```python
from build123d import *

# Parameters (mm, degrees)
SKETCH_1_W             = 35
SKETCH_1_H             = 56.7
EXTRUDE_1_DEPTH        = 12
CHAMFER_1_SIZE         = 2
SKETCH_4_W             = 28
SKETCH_4_H             = 12
EXTRUDE_2_DEPTH        = 35
HOLE_WIZARD_M5_1_D     = 4.2
CHAMFER_2_SIZE         = 2
HOLE_WIZARD_M5_2_D     = 4.2
HOLE_WIZARD_M5_2_DEPTH = 12.4
HOLE_WIZARD_M5_2_TIP   = 1.2618073


with BuildPart() as part:
    # 草图1 → 凸台-拉伸1 (new body)
    with BuildSketch(Plane.XY):
        Rectangle(SKETCH_1_W, SKETCH_1_H)
    extrude(amount=EXTRUDE_1_DEPTH)

    # 倒角1
    chamfer_1_edges = [part.edges().sort_by_distance(p)[0] for p in [
        (-17.5, -28.35, 6),
        (17.5, -28.35, 6),
    ]]
    chamfer(chamfer_1_edges, length=CHAMFER_1_SIZE)

    # 草图4 → 凸台-拉伸2 (add)
    with BuildSketch(Plane.ZY.offset(17.5)):
        with Locations((26, 22.35)):
            Rectangle(SKETCH_4_W, SKETCH_4_H)
    extrude(amount=-EXTRUDE_2_DEPTH)

    # M5 螺纹孔1 (through all)
    with Locations(Plane(origin=(0, 0, 0), x_dir=(-1, 0, 0), z_dir=(0, 0, -1))):
        with Locations((-10, -8.35), (10, -8.35)):
            Hole(HOLE_WIZARD_M5_1_D / 2)

    # 倒角2
    chamfer_2_edges = [part.edges().sort_by_distance(p)[0] for p in [
        (-17.5, 22.35, 40),
        (17.5, 22.35, 40),
    ]]
    chamfer(chamfer_2_edges, length=CHAMFER_2_SIZE)

    # M5 螺纹孔2
    with Locations(Plane(origin=(0, 28.35, 0), x_dir=(1, 0, 0), z_dir=(0, 1, 0))):
        with Locations((-10, -6.5), (10, -6.5), (-10, -31.5), (10, -31.5)):
            Hole(HOLE_WIZARD_M5_2_D / 2, depth=HOLE_WIZARD_M5_2_DEPTH)
            with Locations((0, 0, -(HOLE_WIZARD_M5_2_DEPTH + HOLE_WIZARD_M5_2_TIP / 2))):  # 118° drill point
                Cone(0, HOLE_WIZARD_M5_2_D / 2, HOLE_WIZARD_M5_2_TIP, mode=Mode.SUBTRACT)


solid = part.part
```
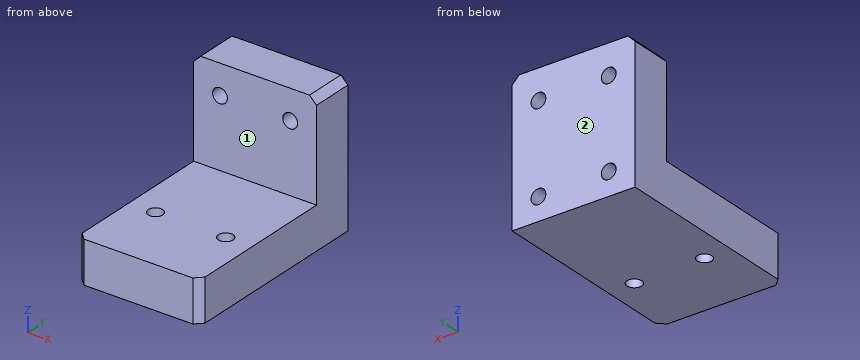
Model file for the job. Use its own axes, mm. Face numbers are marked on the shaded views. A direction names the side the tool comes from. Coordinates: 2 decimals unless noted, no trailing zeros. Loops run counter-clockwise (first coordinate to the right, second up) from the corner with the lowest first, then second, coordinate; pieces in that order, holes last. Notation, with made-up numbers: (67, -10.75) - (100, -10.75) arc R26 ccw to (100, 9.25) - close; hole circle Ø5 at (83.25, -30.5). An arc over 180 degrees is marked (long way). Answer as a JSON object with one key per item and string values. Group by question number.
(1) Cut at A-A (z = 31.5). Give the cut face in (x, y), then the cut area to 3 significant figures.
(2) Cut at B-B (y = -8.35). Give the cut face in (x, z), then the cut area to 3 significant figures.
(3) Cut at D-D (x = -2). Give the cut face in (y, z).
(4) Probe line 1 along Z through (x, y) = (-10, 23); line 2 along Y through (x, z) = (-10, 11.5); line 3 along X through (y, z) = (-8, 8). List the from-to ranges inside material, lowest first.
(5) Flat gauge pins, fed straight in: pin 1 (3.5 mm diameter, centred on x = -10, z = 31.5, fed in from -Y); pin 2 (10 mm diameter, centred on x = -8, z = 35.5, fed in from -Y); pin 3 (4 mm diameter, centred on x = 10, z = 6.5, fed in from +Y); pin 4 (6 mm diameter, centred on x = 14, y = 2.5, fed in from +Z). Where does each tip first touch, or does it go through?
(6) Tool access for the marked faces 1 and 2: list every direction of +Z, -Z, +X, -X, +Y, -Y with a clear straight run to the whole face (end or side of a thin tool).
(7) Cut at C-C (y = 22). Give the cut face in (x, z).
Geometry says:
{
 "1": {"outline": "(-17.5, 16.35) - (-12.1, 16.35) - (-12.1, 28.35) - (-17.5, 28.35) - close; (-7.9, 16.35) - (7.9, 16.35) - (7.9, 28.35) - (-7.9, 28.35) - close; (12.1, 16.35) - (17.5, 16.35) - (17.5, 28.35) - (12.1, 28.35) - close", "area": "319 mm^2"},
 "2": {"outline": "(-17.5, 0) - (-12.1, 0) - (-12.1, 12) - (-17.5, 12) - close; (-7.9, 0) - (7.9, 0) - (7.9, 12) - (-7.9, 12) - close; (12.1, 0) - (17.5, 0) - (17.5, 12) - (12.1, 12) - close", "area": "319 mm^2"},
 "3": {"outline": "(-28.35, 0) - (28.35, 0) - (28.35, 40) - (16.35, 40) - (16.35, 12) - (-28.35, 12) - close"},
 "4": {"line 1": "z = 0 to 4.4, 8.6 to 29.4, 33.6 to 40", "line 2": "y = -28.35 to -10.45, -6.25 to 28.35", "line 3": "x = -17.5 to -12.07, -7.93 to 7.93, 12.07 to 17.5"},
 "5": {"pin 1": "passes through", "pin 2": "stops at y = 16.35", "pin 3": "stops at y = 15.89", "pin 4": "stops at z = 12"},
 "6": {"face 1": "+Z, +X, -X, -Y", "face 2": "+Z, -Z, +X, -X, +Y"},
 "7": {"outline": "(-17.5, 0) - (17.5, 0) - (17.5, 38) - (15.5, 40) - (-15.5, 40) - (-17.5, 38) - close; hole circle Ø4.2 at (-10, 6.5); hole circle Ø4.2 at (-10, 31.5); hole circle Ø4.2 at (10, 6.5); hole circle Ø4.2 at (10, 31.5)"}
}
